```python
from build123d import *

# Parameters (mm, degrees)
SKETCH1_W             = 274
SKETCH1_H             = 90
BOSS_EXTRUDE1_DEPTH   = 5
M5_TAPPED_HOLE1_D     = 4.2
M6_TAPPED_HOLE1_D     = 5
F_6_0MM_BLIND_HOLE1_D = 6
CHAMFER1_SIZE         = 1


with BuildPart() as part:
    # Sketch1 → Boss-Extrude1 (new, symmetric)
    with BuildSketch(Plane.XY):
        Rectangle(SKETCH1_W, SKETCH1_H)
    extrude(amount=BOSS_EXTRUDE1_DEPTH, both=True)

    # M5 Tapped Hole1 (through all)
    with Locations(Plane.XY.offset(5)):
        with Locations((-120, 19), (-120, -19), (120, -19), (120, 19)):
            Hole(M5_TAPPED_HOLE1_D / 2)

    # M6 Tapped Hole1 (through all)
    with Locations(Plane(origin=(0, 0, -5), x_dir=(-1, 0, 0), z_dir=(0, 0, -1))):
        with Locations((112, 35), (112, -35), (-8, -35), (-8, 35)):
            Hole(M6_TAPPED_HOLE1_D / 2)

    # Ø6.0mm blind hole1 (through all)
    with Locations(Plane(origin=(0, 0, -5), x_dir=(-1, 0, 0), z_dir=(0, 0, -1))):
        with Locations((112, 0), (-8, 0)):
            Hole(F_6_0MM_BLIND_HOLE1_D / 2)

    # Chamfer1
    chamfer1_edges = [part.edges().sort_by_distance(p)[0] for p in [
        (137, -45, 0),
        (-137, -45, 0),
        (-137, 45, 0),
        (137, 45, 0),
    ]]
    chamfer(chamfer1_edges, length=CHAMFER1_SIZE)


solid = part.part
```
Source: CAD feature listing. Evaluate the final solid. Frame: model axes, mm. Round coordinates to 2 decimals unless told otherwise and drop trailing zeros. Loops run counter-clockwise (first coordinate to the right, second up) from the corner with the lowest first, then second, coordinate; pieces in that order, holes last. Notation, with made-up numbers: M -27.5,47 L -16.5,47 A30 ccw -16.5,82 Z; hole C 59.25,-22.75 d8. An arc over 180 degrees is marked long. Put each result on its own line as item: value.
(1) Pull-direction query (X, two-part tool) for faces 1 (the face through (-2, 1, -5)), 2 (the face through (10.385, 35.751, 0.07)), 3 (the face through (-137, -1, 0)); classes: released by +X, released by -X, zero draft, split by the parting line, or undercut.
Solutions:
face 1: zero draft
face 2: undercut
face 3: released by -X
(2) Section A-A, the plane y = 35. Return loops of the section in (x, z).
Solutions:
outline: M -137,-5 L -114.5,-5 L -114.5,5 L -137,5 Z; M -109.5,-5 L 5.5,-5 L 5.5,5 L -109.5,5 Z; M 10.5,-5 L 137,-5 L 137,5 L 10.5,5 Z
(3) Section B-B, the plane x = -112. Return loops of the section in (y, z), and give its area (3 significant figures).
Solutions:
outline: M -45,-5 L -37.5,-5 L -37.5,5 L -45,5 Z; M -32.5,-5 L -3,-5 L -3,5 L -32.5,5 Z; M 3,-5 L 32.5,-5 L 32.5,5 L 3,5 Z; M 37.5,-5 L 45,-5 L 45,5 L 37.5,5 Z
area: 740 mm²
(4) Ray query, line 1 (Y direction, x = -121.5, z = -4.5); line 2 (X direction, y = -33, z = -3); line 3 (X direction, y = -1.5, z = -2.5). Return the intervals inside material, ascending. Write a range as [from, to].
Solutions:
line 1: [-45, -20.47], [-17.53, 17.53], [20.47, 45]
line 2: [-137, -113.5], [-110.5, 6.5], [9.5, 137]
line 3: [-137, -114.6], [-109.4, 5.4], [10.6, 137]
(5) Section C-C, the plane y = 0. Return loops of the section in (x, z), and give its area (3 significant figures).
Solutions:
outline: M -137,-5 L -115,-5 L -115,5 L -137,5 Z; M -109,-5 L 5,-5 L 5,5 L -109,5 Z; M 11,-5 L 137,-5 L 137,5 L 11,5 Z
area: 2,620 mm²
(6) First-contact query: pin 1 (6 mm diameter, centred on x = 8, y = 35, fed in from +Z); pin 2 (4.5 mm diameter, centred on x = -112, y = -35, fed in from +Z). Flat tips, straight axial feed; report the tip coordinate or a pass-through.
Solutions:
pin 1: z = 5
pin 2: through
